Could you check a few things on this model? Use its own coordinates, in mm. A direction names the side the tool comes from. Round coordinates to 2 decimals unless told otherwise and drop trailing zeros. Loops run counter-clockwise (first coordinate to the right, second up) from the corner with the lowest first, then second, coordinate; pieces in that order, holes last. Notation, with made-up numbers: (32, -9.75) -> (83, -9.75) arc R13 cw to (83, 15.25) -> close; hole circle Ø7 at (76, 61). An arc over 180 degrees is marked (long way). One line per item, written item: value.
```python
from build123d import *

# Parameters (mm, degrees)
UPRIGHT_PLATE_SKETCH_R          = 10
UPRIGHT_PLATE_DEPTH             = 25
BASE_PLATE_SKETCH_W             = 150
BASE_PLATE_SKETCH_H             = 25
BASE_PLATE_DEPTH                = 120
BASE_PLATE_CORNER_FILLETS_R25_R = 25
BASE_PLATE_HOLES_SKETCH_R       = 10
BASE_PLATE_HOLES_DEPTH          = 206.730406114
WEDGE_SUPPORT_DEPTH             = 60
LUG_PROFILE_CUT_REACH           = 227.051
LUG_PROFILE_SKETCH_R            = 15
LUG_BORE_SKETCH_R               = 15
LUG_BORE_DEPTH                  = 226.05084201
LUG_SLOT_SKETCH_W               = 80
LUG_SLOT_SKETCH_H               = 15
LUG_SLOT_15X20_DEPTH            = 15


with BuildPart() as part:
    # Upright Plate Sketch → Upright Plate (new body)
    with BuildSketch(Plane.XY):
        with BuildLine():
            Line((-60, 45), (60, 45))
            Line((60, 45), (60, -20))
            ThreePointArc((60, -20), (52.67766953, -37.67766953), (35, -45))
            Line((35, -45), (-35, -45))
            ThreePointArc((-35, -45), (-52.67766953, -37.67766953), (-60, -20))
            Line((-60, -20), (-60, 45))
        make_face()
        with Locations((-35, -20)):
            Circle(UPRIGHT_PLATE_SKETCH_R, mode=Mode.SUBTRACT)
        with Locations((35, -20)):
            Circle(UPRIGHT_PLATE_SKETCH_R, mode=Mode.SUBTRACT)
    extrude(amount=-UPRIGHT_PLATE_DEPTH)

    # Base Plate Sketch → Base Plate (add)
    with BuildSketch(Plane(origin=(60, 0, 0), x_dir=(0, 0, -1), z_dir=(1, 0, 0))):
        with Locations((100, 32.5)):
            Rectangle(BASE_PLATE_SKETCH_W, BASE_PLATE_SKETCH_H)
    extrude(amount=-BASE_PLATE_DEPTH)

    # Base Plate Corner Fillets R25
    base_plate_corner_fillets_r25_edges = [part.edges().sort_by_distance(p)[0] for p in [
        (-60, 32.5, -175),
        (60, 32.5, -175),
    ]]
    fillet(base_plate_corner_fillets_r25_edges, radius=BASE_PLATE_CORNER_FILLETS_R25_R)

    # Base Plate Holes Sketch → Base Plate Holes (cut, through all)
    with BuildSketch(Plane(origin=(0, 45, 0), x_dir=(1, 0, 0), z_dir=(0, 1, 0))):
        with Locations(Location((35, 150, 0), (0, 0, 270))):
            Circle(BASE_PLATE_HOLES_SKETCH_R)
        with Locations(Location((-35, 150, 0), (0, 0, 270))):
            Circle(BASE_PLATE_HOLES_SKETCH_R)
    extrude(amount=-BASE_PLATE_HOLES_DEPTH, mode=Mode.SUBTRACT)

    # Wedge Support Sketch → Wedge Support (add, symmetric)
    with BuildSketch(Plane(origin=(0, 0, 0), x_dir=(0, 0, -1), z_dir=(1, 0, 0))):
        Polygon((134.350288425, 45), (67.175144213, 112.175144213), (0, 45), align=None)
    extrude(amount=WEDGE_SUPPORT_DEPTH, both=True)

    # Lug Profile Cut: up to this face of the body (flat: up to its plane)
    lug_profile_cut_end = Plane(part.part.faces().sort_by_distance((0, 45, -154.419772532))[0])
    # Lug Profile Sketch → Lug Profile Cut (cut, up to the picked face)
    with BuildSketch(Plane(origin=(0, 22.5, 22.5), x_dir=(1, 0, 0), z_dir=(0, 0.7071067811865485, 0.7071067811865467)), mode=Mode.PRIVATE) as lug_profile_cut_sk1:
        with BuildLine():
            Line((-40, 31.819805153), (-40, 86.819805153))
            ThreePointArc((-40, 86.819805153), (-28.284271247, 115.104076401), (0, 126.819805153))
            Line((0, 126.819805153), (-60, 126.819805153))
            Line((-60, 126.819805153), (-60, 31.819805153))
            Line((-60, 31.819805153), (-40, 31.819805153))
        make_face()
    lug_profile_cut_tool1 = split(extrude(lug_profile_cut_sk1.sketch, amount=-LUG_PROFILE_CUT_REACH, mode=Mode.PRIVATE), bisect_by=lug_profile_cut_end, keep=Keep.BOTH, mode=Mode.PRIVATE)
    # Lug Profile Sketch → Lug Profile Cut (cut, up to the picked face)
    with BuildSketch(Plane(origin=(0, 22.5, 22.5), x_dir=(1, 0, 0), z_dir=(0, 0.7071067811865485, 0.7071067811865467)), mode=Mode.PRIVATE) as lug_profile_cut_sk2:
        with BuildLine():
            Line((60, 126.819805153), (0, 126.819805153))
            ThreePointArc((0, 126.819805153), (28.284271247, 115.104076401), (40, 86.819805153))
            Line((40, 86.819805153), (40, 31.819805153))
            Line((40, 31.819805153), (60, 31.819805153))
            Line((60, 31.819805153), (60, 126.819805153))
        make_face()
    lug_profile_cut_tool2 = split(extrude(lug_profile_cut_sk2.sketch, amount=-LUG_PROFILE_CUT_REACH, mode=Mode.PRIVATE), bisect_by=lug_profile_cut_end, keep=Keep.BOTH, mode=Mode.PRIVATE)
    # Lug Profile Sketch → Lug Profile Cut (cut, up to the picked face)
    with BuildSketch(Plane(origin=(0, 22.5, 22.5), x_dir=(1, 0, 0), z_dir=(0, 0.7071067811865485, 0.7071067811865467)), mode=Mode.PRIVATE) as lug_profile_cut_sk3:
        with Locations(Location((0, 86.819805153, 0), (0, 0, 270))):
            Circle(LUG_PROFILE_SKETCH_R)
    lug_profile_cut_tool3 = split(extrude(lug_profile_cut_sk3.sketch, amount=-LUG_PROFILE_CUT_REACH, mode=Mode.PRIVATE), bisect_by=lug_profile_cut_end, keep=Keep.BOTH, mode=Mode.PRIVATE)
    add(lug_profile_cut_tool1.solids().sort_by(Axis((-47.101904, 82.761408, -37.761408), (0, -0.7071067811865485, -0.7071067811865467)))[0], mode=Mode.SUBTRACT)
    add(lug_profile_cut_tool2.solids().sort_by(Axis((47.101904, 82.761408, -37.761408), (0, -0.7071067811865485, -0.7071067811865467)))[0], mode=Mode.SUBTRACT)
    add(lug_profile_cut_tool3.solids().sort_by(Axis((0, 83.890873, -38.890873), (0, -0.7071067811865485, -0.7071067811865467)))[0], mode=Mode.SUBTRACT)

    # Lug Bore Sketch → Lug Bore (cut, through all)
    with BuildSketch(Plane(origin=(0, 22.5, 22.5), x_dir=(1, 0, 0), z_dir=(0, 0.7071067811865485, 0.7071067811865467))):
        with Locations(Location((0, 86.819805153, 0), (0, 0, 270))):
            Circle(LUG_BORE_SKETCH_R)
    extrude(amount=-LUG_BORE_DEPTH, mode=Mode.SUBTRACT)

    # Lug Slot Sketch → Lug Slot 15x20 (cut)
    with BuildSketch(Plane(origin=(0, 22.5, 22.5), x_dir=(1, 0, 0), z_dir=(0, 0.7071067811865485, 0.7071067811865467))):
        with Locations((0, 59.319805153)):
            Rectangle(LUG_SLOT_SKETCH_W, LUG_SLOT_SKETCH_H)
    extrude(amount=-LUG_SLOT_15X20_DEPTH, mode=Mode.SUBTRACT)


solid = part.part
```
(1) Please list where these lines run through material, in increasing order: L1, parallel to X at y = 30, z = -150; L2, parallel to Z at x = 36, y = 2; L3, parallel to Y at x = 51, z = -46.
Results below:
L1: x = -60 to -45, -25 to 25, 45 to 60
L2: z = -25 to 0
L3: y = 20 to 45
(2) Imagine slicing it at D-D on y = 41. Give the number of separate pieces and of enclosed holes in the cut face, then the cut area to 3 significant figures.
Results below:
separate pieces: 1
enclosed holes: 3
area: 19,100 mm²
(3) For pin 1 Ø1 at (x, z) = (-1, -71.5) entering from +Y; pin 2 Ø1 at (x, z) = (-44.5, -66) entering from -Y; pin 3 Ø12 at (x, z) = (23, -73.5) entering from +Y; pin 4 Ø16 at (x, y) = (-35, -20) entering from +Z, each with a flat end and sliding along its axis, tell me the tip position at first contact or that it passes through.
Results below:
pin 1: stops at y = 108.33
pin 2: stops at y = 20
pin 3: stops at y = 103.55
pin 4: passes through
(4) Imagine slicing it at C-C on z = -17. Write out the boundary of the cut face in (x, y), then the cut area to 3 significant figures.
Results below:
outline: (-60, -20) arc R25 ccw to (-35, -45) -> (35, -45) arc R25 ccw to (60, -20) -> (60, 45) -> (40, 45) -> (40, 56.28) -> (-40, 56.28) -> (-40, 45) -> (-60, 45) -> close; hole circle Ø20 at (-35, -20); hole circle Ø20 at (35, -20)
area: 10,800 mm²
(5) Imagine slicing it at B-B on x = 7. Write out the boundary of the cut face in (y, z).
Results below:
outline: (-45, -25) -> (20, -25) -> (20, -84.02) -> (74.51, -29.51) -> (69.75, -24.75) -> (59.14, -35.36) -> (48.54, -24.75) -> (59.14, -14.14) -> (45, 0) -> (-45, 0) -> close; (20, -175) -> (45, -175) -> (45, -133.48) -> (111.74, -66.74) -> (93.27, -48.27) -> (20, -121.54) -> close
(6) Imagine slicing it at A-A on x = 32.5. Write out the boundary of the cut face in (y, z), then the cut area to 3 significant figures.
Results below:
outline: (-45, -25) -> (-29.68, -25) -> (-29.68, 0) -> (-45, 0) -> close; (-10.32, -25) -> (20, -25) -> (20, -140.32) -> (45, -140.32) -> (45, -110.76) -> (100.38, -55.38) -> (69.75, -24.75) -> (59.14, -35.36) -> (48.54, -24.75) -> (59.14, -14.14) -> (45, 0) -> (-10.32, 0) -> close; (20, -175) -> (45, -175) -> (45, -159.68) -> (20, -159.68) -> close
area: 7,870 mm²
(7) We'd pull the mould along Z, two halves only. Please class faces 5 (the face through (0, 32, -175)), 6 (the face through (-0.56, 53.913, -19.371)), 7 (the face through (-42.37, -13.24, -12.32)): +Z half, -Z half, draft (parallel to the pull), parting line (faces both ways), or undercut.
Results below:
face 5: -Z half
face 6: undercut
face 7: draft
(8) On a 3-axis mill with a long thin cutter (end or side, diameter ignored), from which of +Z, -Z, +X, -X, +Y, -Y can I reach the whole of each face in a straight line? I mean faces 1 (the face through (-40, 59, -42)), 2 (the face through (1, -12, -25)), 3 (the face through (40, 59, -43)), 4 (the face through (28, 45, -125)). Say none if no direction works.
Results below:
face 1: +Z, -Z, -X, +Y
face 2: -Z, +X, -X, -Y
face 3: +Z, -Z, +X, +Y
face 4: -Z, +Y
